Part model, mm, in its own coordinate system. A direction names the side the tool comes from. Give positions to 0.01 mm unless a question says otherwise; leave off trailing zeros. Write each loop counter-clockwise with the first axis right and the second up, starting at its lowest first coordinate (ties: lowest second). Pieces come first, ordered by that corner, then holes. Notation, with made-up numbers: (6, 58) - (55, 58) arc R21 cw to (55, 95) - close; hole circle Ø5 at (64.25, 53.5). An arc over 180 degrees is marked (long way). Answer in a Markdown table with one row per item. Add a question column.
1. Pull direction Y, two halves, no side cores. Call faces 1 (the flat face through (7, -146, 0)), 2 (the flat face through (2, 175, -2)), 3 (the flat face through (3, -175, -6)): released by +Y, released by -Y, zero draft, split by the parting line, or undercut.
2. Band-saw the part on A-A on y = 40. Write the cut outline in (x, z).
3. Probe line 1 along X through (y, z) = (168.5, 0); line 2 along Y through (x, z) = (6.75, 3.25); line 3 along Z through (x, y) = (-3.75, 42). List the from-to ranges inside material, lowest first.
4. Which spindle directions (+Z, -Z, +X, -X, +Y, -Y) get a long thin tool onto all of the face, cutting with end or side? Do faces 4 (the cylindrical face through (7.932, 2.443, -1.041)), 5 (the flat face through (-7, -146, 0)), 6 (the cylindrical face through (-3.955, -176.232, 5.158)). Say none if no direction does.
5. Drop flat-ended pins along their axis: pin 1 Ø4.5 at (x, z) = (0, 0) entering from +Y; pin 2 Ø2 at (x, y) = (6, 51) entering from -Z (3 decimals); pin 3 Ø4 at (x, y) = (-6.5, -60.5) entering from +Z. Give the stop position or say it passes through.
```python
from build123d import *

# Parameters (mm, degrees)
SKETCH1_R             = 8
BOSS_EXTRUDE1_DEPTH   = 175
CUT_EXTRUDE1_START    = -20
SKETCH8_OUTSIDE_W     = 88.146
SKETCH8_OUTSIDE_H     = 88.146
SKETCH8_OUTSIDE_W_2   = 14
SKETCH8_OUTSIDE_H_2   = 30.19056833
CUT_EXTRUDE1_DEPTH    = 18
SKETCH9_R             = 6.5
BOSS_EXTRUDE2_DEPTH   = 3
M6_TAPPED_HOLE2_D     = 5
M6_TAPPED_HOLE2_DEPTH = 17
M6_TAPPED_HOLE2_TIP   = 1.502151548
CHAMFER1_SIZE         = 0.5
CHAMFER2_SIZE         = 0.5


with BuildPart() as part:
    # Sketch1 → Boss-Extrude1 (new, symmetric)
    with BuildSketch(Plane(origin=(0, 0, 0), x_dir=(1, 0, 0), z_dir=(0, 1, 0))):
        with Locations(Location((0, 0, 0), (0, 0, 270))):
            Circle(SKETCH1_R)
    extrude(amount=BOSS_EXTRUDE1_DEPTH, both=True)

    # Sketch7 → M6 Tapped Hole1 (revolve, cut)
    with BuildSketch(Plane(origin=(0, 175, 0), x_dir=(0, 0, 1), z_dir=(1, 0, 0))):
        Polygon((0, 0), (0, 16.502151548), (2.5, 15), (2.5, 0), align=None)
    m6_tapped_hole1 = revolve(axis=Axis((0, 181.35, 0), (0, -1, 0)), mode=Mode.SUBTRACT)

    # Mirror1: M6 Tapped Hole1 across plane
    add(m6_tapped_hole1.mirror(Plane.ZX), mode=Mode.SUBTRACT)

    # Sketch8 outside → Cut-Extrude1 (cut)
    with BuildSketch(Plane.XZ.offset(175).offset(CUT_EXTRUDE1_START)):
        Rectangle(SKETCH8_OUTSIDE_W, SKETCH8_OUTSIDE_H)
        Rectangle(SKETCH8_OUTSIDE_W_2, SKETCH8_OUTSIDE_H_2, mode=Mode.SUBTRACT)
    extrude(amount=-CUT_EXTRUDE1_DEPTH, mode=Mode.SUBTRACT)

    # Sketch9 → Boss-Extrude2 (add)
    with BuildSketch(Plane.XZ.offset(175)):
        with Locations(Location((0, 0, 0), (0, 0, 270))):
            Circle(SKETCH9_R)
    extrude(amount=BOSS_EXTRUDE2_DEPTH)

    # M6 Tapped Hole2
    with Locations(Plane(origin=(0, -178, 0), x_dir=(-1, 0, 0), z_dir=(0, -1, 0))):
        with Locations((0, 0)):
            Hole(M6_TAPPED_HOLE2_D / 2, depth=M6_TAPPED_HOLE2_DEPTH)
            with Locations((0, 0, -(M6_TAPPED_HOLE2_DEPTH + M6_TAPPED_HOLE2_TIP / 2))):  # 118° drill point
                Cone(0, M6_TAPPED_HOLE2_D / 2, M6_TAPPED_HOLE2_TIP, mode=Mode.SUBTRACT)

    # Chamfer1
    chamfer1_edges = [part.edges().sort_by_distance(p)[0] for p in [
        (0, -175, -8),
        (0, -178, 6.5),
    ]]
    chamfer(chamfer1_edges, length=CHAMFER1_SIZE)

    # Chamfer2
    chamfer2_edges = [part.edges().sort_by_distance(p)[0] for p in [
        (0, 175, -8),
    ]]
    chamfer(chamfer2_edges, length=CHAMFER2_SIZE)


solid = part.part
```
Values:
| question | item | result |
|---|---|---|
| 1 | face 1 | undercut |
| 1 | face 2 | released by +Y |
| 1 | face 3 | released by -Y |
| 2 | outline | circle Ø16 at (0, 0) |
| 3 | line 1 | x = -8 to -2.5, 2.5 to 8 |
| 3 | line 2 | y = -175 to 175 |
| 3 | line 3 | z = -7.07 to 7.07 |
| 4 | face 4 | +Y, -Y |
| 4 | face 5 | +Z, -Z, -X |
| 4 | face 6 | -Y |
| 5 | pin 1 | stops at y = 159.85 |
| 5 | pin 2 | stops at z = -6.245 |
| 5 | pin 3 | stops at z = 6.61 |
